Geometry: final body of the model. Coordinates: model frame, mm. Face numbers are marked on the shaded views. A direction names the side the tool comes from. Give positions to 0.01 mm unless a question says otherwise; leave off trailing zeros. Write each loop counter-clockwise with the first axis right and the second up, starting at its lowest first coordinate (ties: lowest second). Pieces come first, ordered by that corner, then holes. Notation, with made-up numbers: (-27, -19) -> (17, -19) arc R14 cw to (17, 8) -> close; hole circle Ø3 at (51.5, 54). An arc over 180 degrees is marked (long way). Answer as a JSON object with one key per item and string values. Group by question number.
(1) Contact query for flat-ended pins moving along their axis: pin 1 Ø2 at (y, z) = (-13, 74.5) entering from -X; pin 2 Ø1.5 at (x, z) = (13, 13.5) entering from -Y; pin 3 Ø1 at (y, z) = (-22.5, 73.5) entering from +X. Output: stop coordinate, or through.
(2) Set-up query: the marked faces 1, 2, 3 and 4. Return all of +Z, -Z, +X, -X, +Y, -Y with unobstructed straight access to the full face (end or side cutting, diameter ignored); none if empty.
(3) Section query D-D on z = 52.5. Output: boundary loops of the cut face in (x, y), plus the area to 3 significant figures.
(4) Draft query along Y for the marked faces 5, 6, 7 and 8. Return one class per face: +Y half, -Y half, draft (parallel to the pull), parting line (faces both ways), or undercut.
(5) Section query C-C on y = 35. Output: boundary loops of the cut face in (x, z) (3 decimals).
(6) Material intervals for probe 1 along Y at (x, z) = (0, 85.5); probe 2 along Z at (x, y) = (24.5, 17); probe 3 along X at (y, z) = (16.5, 12), sorted ascending.
(7) Section query B-B on z = 6. Output: boundary loops of the cut face in (x, y), plus the area to 3 significant figures.
(8) Section query A-A on y = 0. Output: boundary loops of the cut face in (x, z).
from build123d import *

# Parameters (mm, degrees)
FLANGE_AND_TUBE_PROFILE_SKETCH_R   = 49
FLANGE_AND_TUBE_PROFILE_SKETCH_R_2 = 25
ROUND_FLANGE_98_DEPTH              = 15
SKETCH1_3_R                        = 25
SKETCH1_3_R_2                      = 13
TUBE_BODY_50_DEPTH                 = 90
OVAL_START                         = -15
OVAL_FLANGE_PROFILE_SKETCH_R       = 6
OVAL_FLANGE_PROFILE_SKETCH_R_2     = 25
OVAL_MOUNTING_FLANGE_DEPTH         = 15
SKETCH2_3_R                        = 17.5
OVAL_FLANGE_BORE_CUT_DEPTH         = 30
FLANGE_HOLES_6X_10_D               = 10
FLANGE_HOLES_6X_10_DEPTH           = 15
FLANGE_HOLES_6X_10_CSINK_D         = 10.05
FLANGE_HOLES_6X_10_CSINK_ANGLE     = 90


with BuildPart() as part:
    # Flange and Tube Profile Sketch → Round Flange _98 (new body)
    with BuildSketch(Plane.XY):
        Circle(FLANGE_AND_TUBE_PROFILE_SKETCH_R)
        Circle(FLANGE_AND_TUBE_PROFILE_SKETCH_R_2, mode=Mode.SUBTRACT)
    extrude(amount=ROUND_FLANGE_98_DEPTH)

    # Sketch1_3 → Tube Body _50 (add)
    with BuildSketch(Plane.XY):
        with Locations(Location((0, 0, 0), (0, 0, 180))):
            Circle(SKETCH1_3_R)
        with Locations(Location((0, 0, 0), (0, 0, 180))):
            Circle(SKETCH1_3_R_2, mode=Mode.SUBTRACT)
    extrude(amount=TUBE_BODY_50_DEPTH)

    # Oval Flange Profile Sketch → Oval Mounting Flange (add)
    with BuildSketch(Plane.XY.offset(90).offset(OVAL_START)):
        with BuildLine():
            Line((14.309088021, -54.5), (28.618176043, -9))
            ThreePointArc((28.618176043, -9), (30, 0), (28.618176043, 9))
            Line((28.618176043, 9), (14.309088021, 54.5))
            ThreePointArc((14.309088021, 54.5), (0, 65), (-14.309088021, 54.5))
            Line((-14.309088021, 54.5), (-28.618176043, 9))
            ThreePointArc((-28.618176043, 9), (-30, 0), (-28.618176043, -9))
            Line((-28.618176043, -9), (-14.309088021, -54.5))
            ThreePointArc((-14.309088021, -54.5), (0, -65), (14.309088021, -54.5))
        make_face()
        with Locations((0, -50)):
            Circle(OVAL_FLANGE_PROFILE_SKETCH_R, mode=Mode.SUBTRACT)
        with Locations((0, 50)):
            Circle(OVAL_FLANGE_PROFILE_SKETCH_R, mode=Mode.SUBTRACT)
        with Locations(Location((0, 0, 0), (0, 0, 180))):
            Circle(OVAL_FLANGE_PROFILE_SKETCH_R_2, mode=Mode.SUBTRACT)
    extrude(amount=OVAL_MOUNTING_FLANGE_DEPTH)

    # Sketch2_3 → Oval Flange Bore Cut (cut)
    with BuildSketch(Plane.XY.offset(90)):
        Circle(SKETCH2_3_R)
    extrude(amount=-OVAL_FLANGE_BORE_CUT_DEPTH, mode=Mode.SUBTRACT)

    # Flange Holes 6x_10
    with Locations(Plane.XY.offset(15)):
        with Locations((-30.310889132, 17.5), (0, 35), (30.310889132, 17.5), (30.310889132, -17.5), (0, -35), (-30.310889132, -17.5)):
            CounterSinkHole(FLANGE_HOLES_6X_10_D / 2, FLANGE_HOLES_6X_10_CSINK_D / 2, depth=FLANGE_HOLES_6X_10_DEPTH, counter_sink_angle=FLANGE_HOLES_6X_10_CSINK_ANGLE)


solid = part.part
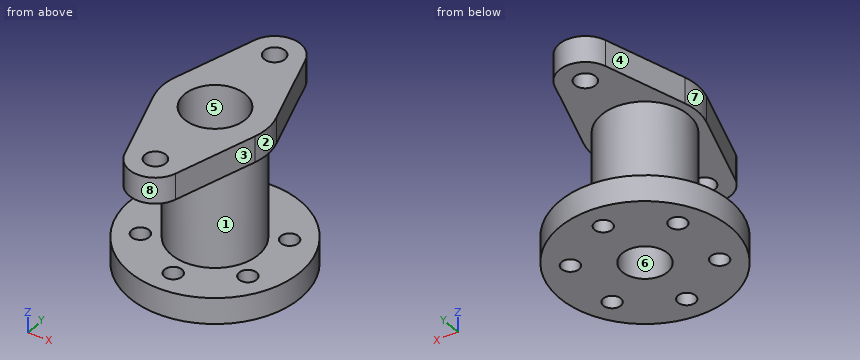
Answer list:
{
 "1": {"pin 1": "x = -27.63", "pin 2": "y = -47.44", "pin 3": "x = 11.87"},
 "2": {"face 1": "none", "face 2": "+Z, +X", "face 3": "+Z, +X, -Y", "face 4": "+Z, -X, +Y"},
 "3": {"outline": "circle Ø50 at (0, 0); hole circle Ø26 at (0, 0)", "area": "1,430 mm2"},
 "4": {"face 5": "undercut", "face 6": "undercut", "face 7": "parting line", "face 8": "-Y half"},
 "5": {"outline": "(-34.293, 0) -> (-5, 0) -> (-5, 14.975) -> (-5.025, 15) -> (-34.293, 15) -> close; (-20.442, 75) -> (20.442, 75) -> (20.442, 90) -> (-20.442, 90) -> close; (5, 0) -> (34.293, 0) -> (34.293, 15) -> (5.025, 15) -> (5, 14.975) -> close"},
 "6": {"probe 1": "-65 to -56, -44 to -17.5, 17.5 to 44, 56 to 65", "probe 2": "0 to 15, 75 to 90", "probe 3": "-46.14 to -35.21, -25.41 to 25.41, 35.21 to 46.14"},
 "7": {"outline": "circle Ø98 at (0, 0); hole circle Ø10 at (-30.31, -17.5); hole circle Ø10 at (-30.31, 17.5); hole circle Ø26 at (0, 0); hole circle Ø10 at (0, -35); hole circle Ø10 at (0, 35); hole circle Ø10 at (30.31, -17.5); hole circle Ø10 at (30.31, 17.5)", "area": "6,540 mm2"},
 "8": {"outline": "(-49, 0) -> (-13, 0) -> (-13, 60) -> (-17.5, 60) -> (-17.5, 90) -> (-30, 90) -> (-30, 75) -> (-25, 75) -> (-25, 15) -> (-49, 15) -> close; (13, 0) -> (49, 0) -> (49, 15) -> (25, 15) -> (25, 75) -> (30, 75) -> (30, 90) -> (17.5, 90) -> (17.5, 60) -> (13, 60) -> close"}
}
